Read the model definition and answer for the solid it produces. Units are mm, in the model's axes. Face numbers are marked on the shaded views. A direction names the side the tool comes from. Give positions to 0.01 mm unless a question says otherwise; leave off trailing zeros. Loops run counter-clockwise (first coordinate to the right, second up) from the corner with the lowest first, then second, coordinate; pieces in that order, holes last. Notation, with made-up numbers: (-15.5, 49) - (7.5, 49) arc R22 cw to (7.5, 79) - close; hole circle Ø8 at (25, 44.25). An arc over 180 degrees is marked (long way). Write each question's results on one line, items separated by ' | '. Start each with the question number.
Q1. The part is cut by section B-B, the plane z = 37. Write down the section's boundary in (x, y).
Q2. For the marked faces 1 and 2, determine the directions among +Z, -Z, +X, -X, +Y, -Y from which every point of the face is accessible in a straight line to the end or side of a thin tool.
Q3. The part is cut by section A-A, the plane y = 7.75. Write down the section's boundary in (x, z), plus the area to 3 significant figures.
Q4. Given pin 1 (9 mm diameter, centred on y = 7.75, z = 180, fed in from -X); pin 2 (8 mm diameter, centred on x = -34.5, z = 94, fed in from -Y); pin 3 (8 mm diameter, centred on y = 3, z = 99, fed in from -X), each flat-ended and moving along its own axis, determine where each tip first touches the part or whether it passes through.
Q5. Find the intervals of material crossed by line 1 (Z direction, x = -13, y = 7.5); line 2 (Y direction, x = -10, z = 40); line 3 (X direction, y = 15.5, z = 60.5), in increasing order. Write a range as from..to.
Q6. The part is cut by section D-D, the plane z = 82. Write down the section's boundary in (x, y).
Q7. The part is cut by section C-C, the plane x = -43. Write down the section's boundary in (y, z).
```python
from build123d import *

# Parameters (mm, degrees)
EXTRUDE_1_DEPTH     = 220
SKETCH_2_R          = 10
CUT_EXTRUDE_1_DEPTH = 24
SKETCH_3_R          = 10
CUT_EXTRUDE_2_DEPTH = 24
SKETCH_4_R          = 7.332886018
SKETCH_4_R_2        = 7.301331484
SKETCH_4_R_3        = 6.603217824
CUT_EXTRUDE_3_DEPTH = 10
CUT_EXTRUDE_START   = -45
SKETCH_5_R          = 7.332886018
SKETCH_5_R_2        = 7.301331484
SKETCH_5_R_3        = 6.603217824
CUT_EXTRUDE_4_DEPTH = 45


with BuildPart() as part:
    # 草图1 → 凸台-拉伸1 (new body)
    with BuildSketch(Plane.XY):
        Polygon((-55.555555556, 26.25), (-5.555555556, 26.25), (-5.555555556, -1.75), (-15.555555556, -1.75), (-15.555555556, 17.25), (-55.555555556, 17.25), align=None)
    extrude(amount=EXTRUDE_1_DEPTH)

    # 草图2 → 切除-拉伸1 (cut)
    with BuildSketch(Plane(origin=(982.792188559, 17.25, -600.126281628), x_dir=(0.9997402704834758, 0, 0.022790163966647386), z_dir=(0, -1, 0))):
        with Locations(Location((-1000.30321436, 803.168334002, 0), (0, 0, 358.694106729))):
            Circle(SKETCH_2_R)
        with Locations(Location((-1001.898940295, 733.168334002, 0), (0, 0, 358.694106729))):
            Circle(SKETCH_2_R)
        with Locations(Location((-1003.49466623, 663.168334002, 0), (0, 0, 358.694106729))):
            Circle(SKETCH_2_R)
        with Locations((-915.325705826, 801.212988999)):
            Circle(SKETCH_2_R)
        with Locations((-916.921431761, 731.212988999)):
            Circle(SKETCH_2_R)
        with Locations((-918.516743239, 661.231170065)):
            Circle(SKETCH_2_R)
    extrude(amount=-CUT_EXTRUDE_1_DEPTH, mode=Mode.SUBTRACT)

    # 草图3 → 切除-拉伸2 (cut)
    with BuildSketch(Plane(origin=(-968.90329967, 17.25, 820.126281628), x_dir=(-0.9997402704834758, 0, -0.022790163966647077), z_dir=(0, -1, 0))):
        with Locations((-1000.30321436, 803.168334002)):
            Circle(SKETCH_3_R)
        with Locations((-1001.898940295, 733.168334002)):
            Circle(SKETCH_3_R)
        with Locations((-1003.49466623, 663.168334002)):
            Circle(SKETCH_3_R)
        with Locations((-915.325705826, 801.212988999)):
            Circle(SKETCH_3_R)
        with Locations((-916.921431761, 731.212988999)):
            Circle(SKETCH_3_R)
        with Locations((-918.516743239, 661.231170065)):
            Circle(SKETCH_3_R)
    extrude(amount=-CUT_EXTRUDE_2_DEPTH, mode=Mode.SUBTRACT)

    # 草图4 → 切除-拉伸3 (cut)
    with BuildSketch(Plane(origin=(-15.555555556, -796.892477777, -600.126281629), x_dir=(0, -1, 0), z_dir=(-1, 0, 0))):
        with Locations(Location((-804.642477777, 640.126281628, 0), (0, 0, 90))):
            Circle(SKETCH_4_R)
        with Locations(Location((-804.642477777, 710.126281628, 0), (0, 0, 90))):
            Circle(SKETCH_4_R_2)
        with Locations(Location((-804.642477777, 780.126281628, 0), (0, 0, 90))):
            Circle(SKETCH_4_R_3)
    extrude(amount=-CUT_EXTRUDE_3_DEPTH, mode=Mode.SUBTRACT)

    # 草图5 → 切除-拉伸4 (cut)
    with BuildSketch(Plane(origin=(29.444444444, -796.892477777, 820.126281629), x_dir=(0, -1, 0), z_dir=(1, 0, 0)).offset(CUT_EXTRUDE_START)):
        with Locations(Location((-804.642477777, 640.126281628, 0), (0, 0, 90))):
            Circle(SKETCH_5_R)
        with Locations(Location((-804.642477777, 710.126281628, 0), (0, 0, 270))):
            Circle(SKETCH_5_R_2)
        with Locations((-804.642477777, 780.126281628)):
            Circle(SKETCH_5_R_3)
    extrude(amount=CUT_EXTRUDE_4_DEPTH, mode=Mode.SUBTRACT)


solid = part.part
```
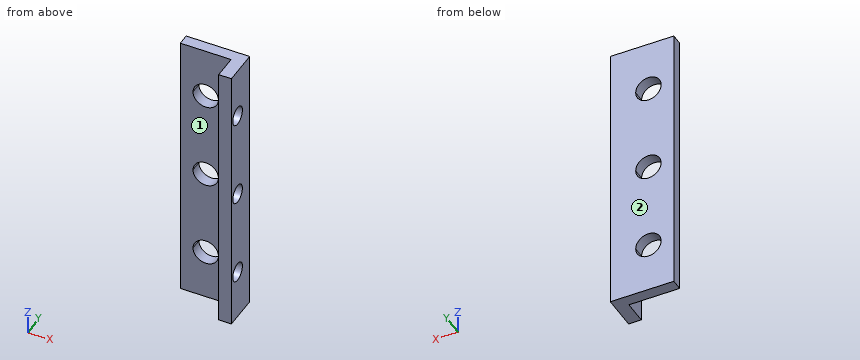
Check sheet entries:
1) outline: (-55.56, 17.25) - (-45.1, 17.25) - (-45.1, 26.25) - (-55.56, 26.25) - close; (-26.01, 17.25) - (-15.56, 17.25) - (-15.56, 14.44) - (-5.56, 14.44) - (-5.56, 26.25) - (-26.01, 26.25) - close; (-15.56, -1.75) - (-5.56, -1.75) - (-5.56, 1.06) - (-15.56, 1.06) - close
2) face 1: +Z, -Z, -X, -Y | face 2: +Z, -Z, +X, -X, +Y
3) outline: (-15.56, 0) - (-5.56, 0) - (-5.56, 32.67) - (-15.56, 32.67) - close; (-15.56, 47.33) - (-5.56, 47.33) - (-5.56, 102.7) - (-15.56, 102.7) - close; (-15.56, 117.3) - (-5.56, 117.3) - (-5.56, 172.67) - (-15.56, 172.67) - close; (-15.56, 187.33) - (-5.56, 187.33) - (-5.56, 220) - (-15.56, 220) - close | area: 1,760 mm^2
4) pin 1: passes through | pin 2: stops at y = 17.25 | pin 3: stops at x = -15.56
5) line 1: z = 0..32.67, 47.33..102.7, 117.3..172.67, 187.33..220 | line 2: y = -1.75..0.42, 15.08..26.25 | line 3: x = -15.56..-5.56
6) outline: (-55.56, 17.25) - (-15.56, 17.25) - (-15.56, -1.75) - (-5.56, -1.75) - (-5.56, 26.25) - (-55.56, 26.25) - close
7) outline: (17.25, 0) - (26.25, 0) - (26.25, 33.3) - (17.25, 33.3) - close; (17.25, 46.68) - (26.25, 46.68) - (26.25, 103.32) - (17.25, 103.32) - close; (17.25, 116.7) - (26.25, 116.7) - (26.25, 173.32) - (17.25, 173.32) - close; (17.25, 186.71) - (26.25, 186.71) - (26.25, 220) - (17.25, 220) - close
